Geometry: see drawing. Coordinates: mm, zero at the bounding-box minimum. Give positions to 0.01 mm unless a question says otherwise; leave off trailing zeros. Order: outer loops, then holes, each group sorted by start corner. A loop starts at its lowest first (then second) coordinate and runs counter-clockwise, first axis right, second up. Notation, with made-up numbers: (68.5, 80) - (112.5, 80) arc R12 cw to (112.5, 87) - close; hole circle Ø8 at (73, -17). An arc over 180 degrees is marked (long way). One line per question, with ' | ' between items. Start each with the question number.
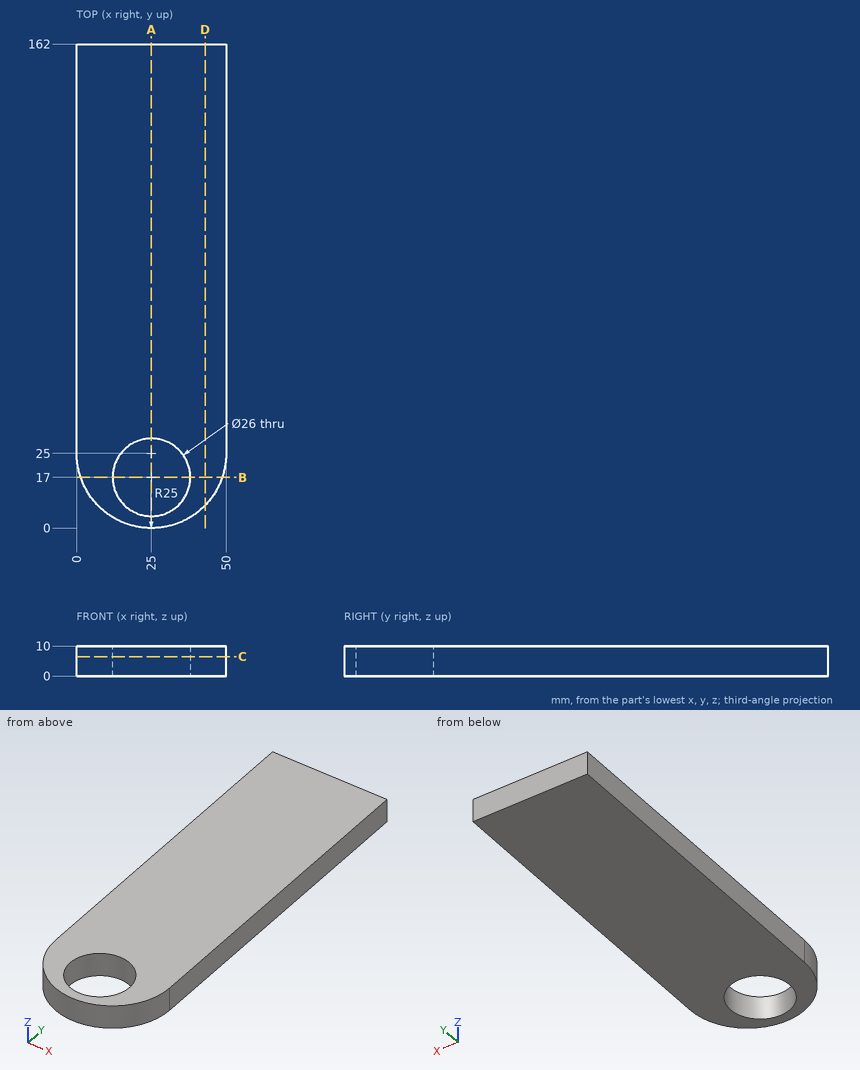
(1) Cut plane C-C, the plane z = 6.5. Return the cut outline in (x, y).
(2) Contact query for flat-ended pins moving along their axis: P1, Ø1, axis at x = 19, z = 3.5, coming from the -Y side; P2, Ø1.5, axis at x = 15.5, z = 4.5, coming from the -Y side. Output: stop coordinate, or through.
(3) Cut plane A-A, the plane x = 25. Return the cut outline in (y, z).
(4) Cut plane B-B, the plane y = 17. Return the cut outline in (x, z), plus the area to 3 significant figures.
(5) Material intervals for line 1 along Y through (x, z) = (25, 7.75); line 2 along X through (y, z) = (23.5, 6.75); line 3 along X through (y, z) = (14.5, 8), sorted ascending. Write a range as from..to.
(6) Cut plane D-D, the plane x = 43. Return the cut outline in (y, z), plus the area to 3 significant figures.
Results are:
1) outline: (0, 25) arc R25 ccw to (50, 25) - (50, 162) - (0, 162) - close; hole circle Ø26 at (25, 17)
2) P1: y = 0.61 | P2: y = 1.58
3) outline: (0, 0) - (4, 0) - (4, 10) - (0, 10) - close; (30, 0) - (162, 0) - (162, 10) - (30, 10) - close
4) outline: (1.31, 0) - (12, 0) - (12, 10) - (1.31, 10) - close; (38, 0) - (48.69, 0) - (48.69, 10) - (38, 10) - close | area: 214 mm2
5) line 1: 0..4, 30..162 | line 2: 0.05..13.74, 36.26..49.95 | line 3: 2.31..12.24, 37.76..47.69
6) outline: (7.65, 0) - (162, 0) - (162, 10) - (7.65, 10) - close | area: 1,540 mm2
